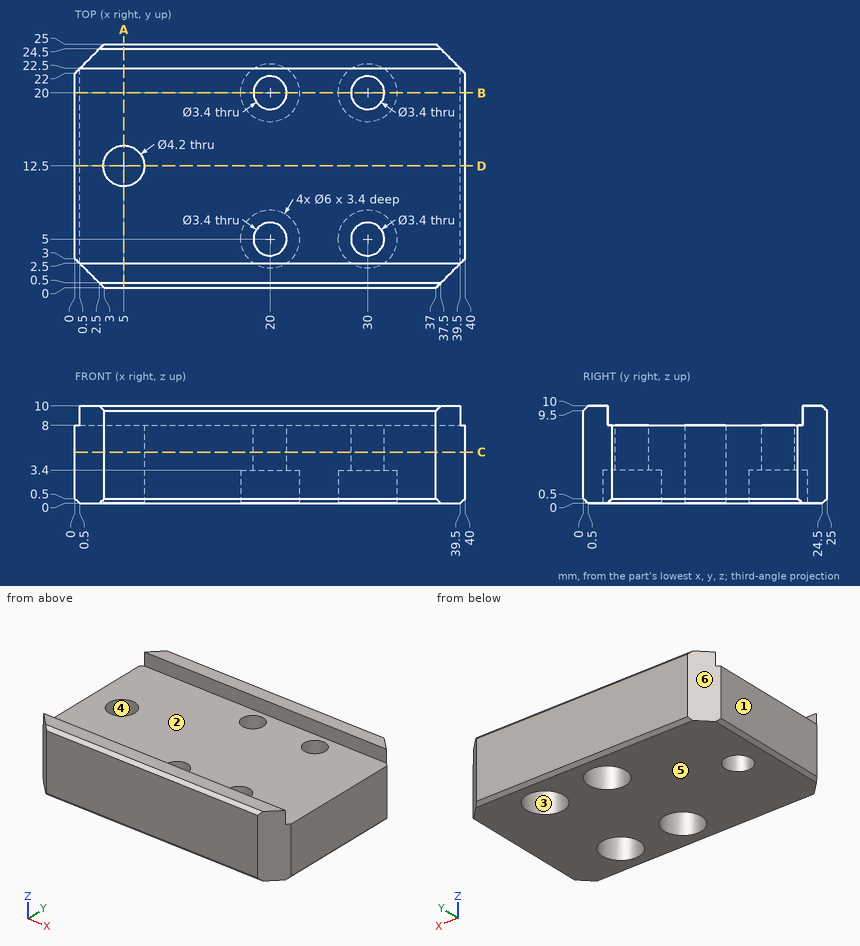
For this review, use the dimensioned drawing (mm, ordinates from the lowest corner) and the shaded views. A direction names the side the tool comes from. Coordinates: 2 decimals unless noted, no trailing zeros. Loops run counter-clockwise (first coordinate to the right, second up) from the corner with the lowest first, then second, coordinate; pieces in that order, holes last.
1. For the marked faces 1, 2 and 3, list the 3-axis set-ups (+Z, -Z, +X, -X, +Y, -Y) from which the entire face can be reached by the end or side of a thin tool; tool diameter is ignored.
2. Add section A-A, the plane x = 5. Give the boundary of the cut face in (y, z).
3. Add section B-B, the plane y = 20. Give the boundary of the cut face in (x, z), then the cut area to 3 significant figures.
4. Mouldability with a two-part tool opening along Y and no side actions: class the marked faces 4, 5 and 6 as +Y half, -Y half, draft (parallel to the pull), parting line (faces both ways), or undercut.
5. For line 1 (Y direction, x = 8, z = 9.25); line 2 (Y direction, x = 20, z = 5.7); line 3 (Y direction, x = 30.5, z = 6.75), list the stretches that pass through material, from the lowest coordinate up.
6. Insertion check: P1, Ø4, axis at x = 20, y = 5, coming from the +Z side; P2, Ø5.5, axis at x = 20, y = 5, coming from the -Z side; P3, Ø2, axis at x = 30, y = 20, coming from the -Z side. Each pin has a flat end and moves straight along its axis. Give the tip position at first contact, or say it passes through.
7. Add section C-C, the plane z = 5.25. Give the boundary of the cut face in (x, y), then the cut area to 3 significant figures.
8. Add section D-D, the plane y = 12.5. Give the boundary of the cut face in (x, z), then the cut area to 3 significant figures.
Result:
1. face 1: +Z, -Z, -X, +Y, -Y
1. face 2: +Z, +X, -X
1. face 3: -Z
2. outline: (0, 0.5) - (0.5, 0) - (10.4, 0) - (10.4, 8) - (2.5, 8) - (2.5, 10) - (0.5, 10) - (0, 9.5) - close; (14.6, 0) - (24.5, 0) - (25, 0.5) - (25, 9.5) - (24.5, 10) - (22.5, 10) - (22.5, 8) - (14.6, 8) - close
3. outline: (0, 0.5) - (0.5, 0) - (17, 0) - (17, 3.4) - (18.3, 3.4) - (18.3, 8) - (0, 8) - close; (21.7, 3.4) - (23, 3.4) - (23, 0) - (27, 0) - (27, 3.4) - (28.3, 3.4) - (28.3, 8) - (21.7, 8) - close; (31.7, 3.4) - (33, 3.4) - (33, 0) - (39.5, 0) - (40, 0.5) - (40, 8) - (31.7, 8) - close
3. area: 248 mm2
4. face 4: undercut
4. face 5: draft
4. face 6: +Y half
5. line 1: y = 0 to 2.5, 22.5 to 25
5. line 2: y = 0 to 3.3, 6.7 to 18.3, 21.7 to 25
5. line 3: y = 0 to 3.38, 6.62 to 18.38, 21.62 to 25
6. P1: stops at z = 8
6. P2: stops at z = 3.4
6. P3: passes through
7. outline: (0, 3) - (3, 0) - (37, 0) - (40, 3) - (40, 22) - (37, 25) - (3, 25) - (0, 22) - close; hole circle Ø4.2 at (5, 12.5); hole circle Ø3.4 at (20, 5); hole circle Ø3.4 at (20, 20); hole circle Ø3.4 at (30, 5); hole circle Ø3.4 at (30, 20)
7. area: 932 mm2
8. outline: (0, 0.5) - (0.5, 0) - (2.9, 0) - (2.9, 8) - (0, 8) - close; (7.1, 0) - (39.5, 0) - (40, 0.5) - (40, 8) - (7.1, 8) - close
8. area: 286 mm2
